from build123d import *

# Parameters (mm, degrees)
SKETCH1_W                                            = 22
SKETCH1_H                                            = 8
BOSS_EXTRUDE1_DEPTH                                  = 7
CUT_EXTRUDE1_DEPTH                                   = 5.8
CHAMFER1_SIZE                                        = 1
HOLE_SIZE_PER_SOCKET_HEAD_CAP_SCREW_TYPE_D           = 2.9
HOLE_SIZE_PER_SOCKET_HEAD_CAP_SCREW_TYPE_CBORE_D     = 5
HOLE_SIZE_PER_SOCKET_HEAD_CAP_SCREW_TYPE_CBORE_DEPTH = 2.9


with BuildPart() as part:
    # Sketch1 → Boss-Extrude1 (new body)
    with BuildSketch(Plane.XY):
        Rectangle(SKETCH1_W, SKETCH1_H)
    extrude(amount=BOSS_EXTRUDE1_DEPTH)

    # Sketch3 → Cut-Extrude1 (cut)
    with BuildSketch(Plane.XY.offset(7)):
        with BuildLine():
            Line((-3, 2), (-1.75, 2))
            Line((-1.75, 2), (-1.75, 4))
            Line((-1.75, 4), (1.75, 4))
            Line((1.75, 4), (1.75, 2))
            Line((1.75, 2), (3, 2))
            ThreePointArc((3, 2), (5, 0), (3, -2))
            Line((3, -2), (1.75, -2))
            Line((1.75, -2), (1.75, -4))
            Line((1.75, -4), (-1.75, -4))
            Line((-1.75, -4), (-1.75, -2))
            Line((-1.75, -2), (-3, -2))
            ThreePointArc((-3, -2), (-5, 0), (-3, 2))
        make_face()
    extrude(amount=-CUT_EXTRUDE1_DEPTH, mode=Mode.SUBTRACT)

    # Chamfer1
    chamfer1_edges = [part.edges().sort_by_distance(p)[0] for p in [
        (11, -4, 3.5),
        (-11, -4, 3.5),
        (-11, 4, 3.5),
        (11, 4, 3.5),
    ]]
    chamfer(chamfer1_edges, length=CHAMFER1_SIZE)

    # Hole size per socket head cap screw type 1 (through all)
    with Locations(Plane.XY.offset(7)):
        with Locations((-8, 0), (8, 0)):
            CounterBoreHole(HOLE_SIZE_PER_SOCKET_HEAD_CAP_SCREW_TYPE_D / 2, HOLE_SIZE_PER_SOCKET_HEAD_CAP_SCREW_TYPE_CBORE_D / 2, HOLE_SIZE_PER_SOCKET_HEAD_CAP_SCREW_TYPE_CBORE_DEPTH)


solid = part.part
Source: CAD feature listing. Evaluate the final solid. Frame: model axes, mm. A direction names the side the tool comes from. Give positions to 0.01 mm unless a question says otherwise; leave off trailing zeros. Write each loop counter-clockwise with the first axis right and the second up, starting at its lowest first coordinate (ties: lowest second). Pieces come first, ordered by that corner, then holes. Notation, with made-up numbers: (-34.5, 89) -> (1.5, 89) arc R19 ccw to (1.5, 120) -> close; hole circle Ø11 at (-18, 10). An arc over 180 degrees is marked (long way). Write item = value, one per line.
Q1. Mould query, pull axis X, two halves, no side actions, for faces 4 (the face through (-5, 0, 4)), 5 (the face through (2, 2, 4)), 6 (the face through (-10.5, 3.5, 3.5)), 7 (the face through (-2, -4, 3)). Classes: +X half, -X half, draft (parallel to the pull), parting line (faces both ways), or undercut.
Here are the results:
face_4 = undercut
face_5 = undercut
face_6 = -X half
face_7 = draft
Q2. Reachability of faces 1 (the face through (-2, 2, 4)), 2 (the face through (1.75, -3, 4)), 3 (the face through (11, 0, 3)) from +Z, -Z, +X, -X, +Y, -Y: full face, straight path, thin tool, end or side. Return the list, or none.
Here are the results:
face_1 = +Z
face_2 = +Z, +Y, -Y
face_3 = +Z, -Z, +X, +Y, -Y
Q3. Cut plane B-B on x = -8. Return loops of the section in (y, z), then the cut area to 3 significant figures.
Here are the results:
outline = (-4, 0) -> (-1.45, 0) -> (-1.45, 4.1) -> (-2.5, 4.1) -> (-2.5, 7) -> (-4, 7) -> close; (1.45, 0) -> (4, 0) -> (4, 7) -> (2.5, 7) -> (2.5, 4.1) -> (1.45, 4.1) -> close
area = 29.6 mm²
Q4. Cut plane C-C on y = 0. Return loops of the section in (x, z), then the cut area to 3 significant figures.
Here are the results:
outline = (-11, 0) -> (-9.45, 0) -> (-9.45, 4.1) -> (-10.5, 4.1) -> (-10.5, 7) -> (-11, 7) -> close; (-6.55, 0) -> (6.55, 0) -> (6.55, 4.1) -> (5.5, 4.1) -> (5.5, 7) -> (5, 7) -> (5, 1.2) -> (-5, 1.2) -> (-5, 7) -> (-5.5, 7) -> (-5.5, 4.1) -> (-6.55, 4.1) -> close; (9.45, 0) -> (11, 0) -> (11, 7) -> (10.5, 7) -> (10.5, 4.1) -> (9.45, 4.1) -> close
area = 43.2 mm²
Q5. Cut plane A-A on z = 3. Return loops of the section in (x, y).
Here are the results:
outline = (-11, -3) -> (-10, -4) -> (-1.75, -4) -> (-1.75, -2) -> (-3, -2) arc R2 cw to (-3, 2) -> (-1.75, 2) -> (-1.75, 4) -> (-10, 4) -> (-11, 3) -> close; (1.75, -4) -> (10, -4) -> (11, -3) -> (11, 3) -> (10, 4) -> (1.75, 4) -> (1.75, 2) -> (3, 2) arc R2 cw to (3, -2) -> (1.75, -2) -> close; hole circle Ø2.9 at (-8, 0); hole circle Ø2.9 at (8, 0)
Q6. Cut plane D-D on z = 6. Return loops of the section in (x, y), then the cut area to 3 significant figures.
Here are the results:
outline = (-11, -3) -> (-10, -4) -> (-1.75, -4) -> (-1.75, -2) -> (-3, -2) arc R2 cw to (-3, 2) -> (-1.75, 2) -> (-1.75, 4) -> (-10, 4) -> (-11, 3) -> close; (1.75, -4) -> (10, -4) -> (11, -3) -> (11, 3) -> (10, 4) -> (1.75, 4) -> (1.75, 2) -> (3, 2) arc R2 cw to (3, -2) -> (1.75, -2) -> close; hole circle Ø5 at (-8, 0); hole circle Ø5 at (8, 0)
area = 84.2 mm²
Q7. Line query: line 1 (X direction, y = 0.5, z = 2); line 2 (X direction, y = 2.5, z = 1.75); line 3 (Y direction, x = 8, z = 2.3). Output: solid intervals per line, ascending. Write a range as from..to.
Here are the results:
line_1 = -11..-9.36, -6.64..-4.94, 4.94..6.64, 9.36..11
line_2 = -11..-1.75, 1.75..11
line_3 = -4..-1.45, 1.45..4
Q8. First-contact query: pin 1 (2.5 mm diameter, centred on x = -8, y = 0, fed in from -Z); pin 2 (4.5 mm diameter, centred on x = 8, y = 0, fed in from +Z); pin 3 (0.6 mm diameter, centred on y = -3.5, z = 5.5, fed in from -X). Flat tips, straight axial feed; report the tip coordinate or a pass-through.
Here are the results:
pin_1 = through
pin_2 = 4.1
pin_3 = -10.8
